from build123d import *

# Parameters (mm, degrees)
SKETCH1_W           = 484
SKETCH1_H           = 378
BOSS_EXTRUDE1_DEPTH = 189
SKETCH2_W           = 318
SKETCH2_H           = 179
CUT_EXTRUDE1_DEPTH  = 553.899629228
SKETCH3_R           = 2.25
SKETCH3_R_2         = 39.056616246
CUT_EXTRUDE2_DEPTH  = 361.563447953


with BuildPart() as part:
    # Sketch1 → Boss-Extrude1 (new body)
    with BuildSketch(Plane(origin=(0, 0, 0), x_dir=(1, 0, 0), z_dir=(0, 1, 0))):
        Rectangle(SKETCH1_W, SKETCH1_H)
    extrude(amount=BOSS_EXTRUDE1_DEPTH)

    # Sketch2 → Cut-Extrude1 (cut, through all)
    with BuildSketch(Plane.ZY.offset(242)):
        with Locations((0, 89.5)):
            Rectangle(SKETCH2_W, SKETCH2_H)
    extrude(amount=-CUT_EXTRUDE1_DEPTH, mode=Mode.SUBTRACT)

    # Sketch3 → Cut-Extrude2 (cut, through all)
    with BuildSketch(Plane(origin=(0, 189, 0), x_dir=(1, 0, 0), z_dir=(0, 1, 0))):
        with Locations(Location((-89, -100, 0), (0, 0, 270))):
            Circle(SKETCH3_R)
        with Locations(Location((89, -100, 0), (0, 0, 270))):
            Circle(SKETCH3_R)
        with Locations(Location((-89, 100, 0), (0, 0, 270))):
            Circle(SKETCH3_R)
        with Locations(Location((89, 100, 0), (0, 0, 270))):
            Circle(SKETCH3_R)
        with Locations(Location((0, 0, 0), (0, 0, 270))):
            Circle(SKETCH3_R_2)
    extrude(amount=-CUT_EXTRUDE2_DEPTH, mode=Mode.SUBTRACT)


solid = part.part
Here's how the part is built. I have some questions about the finished solid (model axes, mm). A direction names the side the tool comes from. Coordinates: 2 decimals unless noted, no trailing zeros. Write each loop counter-clockwise with the first axis right and the second up, starting at its lowest first coordinate (ties: lowest second). Pieces come first, ordered by that corner, then holes.
1) If I drill on line 1 (X direction, y = 182, z = -100); line 2 (Z direction, x = -96, y = 79.5); line 3 (Y direction, x = -42.5, z = -84.5), over which ranges is the centre line in solid material (lowest first)?
Filled in:
line 1: x = -242 to -91.25, -86.75 to 86.75, 91.25 to 242
line 2: z = -189 to -159, 159 to 189
line 3: y = 179 to 189
2) If we section it at D-D (z = -92): List the corners of the cut face in (x, y) for me.
Filled in:
outline: (-242, 179) - (242, 179) - (242, 189) - (-242, 189) - close
3) If we section it at A-A (z = 0): List the corners of the cut face in (x, y) for me, plus the area to 3 significant figures.
Filled in:
outline: (-242, 179) - (-39.06, 179) - (-39.06, 189) - (-242, 189) - close; (39.06, 179) - (242, 179) - (242, 189) - (39.06, 189) - close
area: 4,060 mm2
4) If we section it at B-B (y = 48): List the corners of the cut face in (x, z) for me.
Filled in:
outline: (-242, -189) - (242, -189) - (242, -159) - (-242, -159) - close; (-242, 159) - (242, 159) - (242, 189) - (-242, 189) - close
5) I'm going to push a flat-ended pin straight in: pin 1 (6 mm diameter, centred on x = 19.5, z = -108, fed in from -Y). Where does the tip first touch, or does it pass through?
Filled in:
pin 1: stops at y = 179
6) Thinking about a two-plate mould opening in Z: for faces 3 (the face through (-3, 93, -189)), 4 (the face through (-3, 0, 174)), 5 (the face through (-23.77, 184.07, -30.99)), which applies, +Z half, -Z half, draft (parallel to the pull), parting line (faces both ways), or undercut?
Filled in:
face 3: -Z half
face 4: draft
face 5: undercut
7) Which directions (+Z, -Z, +X, -X, +Y, -Y) give clear straight access to the entire face, cutting with the end or side of a thin tool? Please do faces 1 (the face through (-242, 185, 1)), 2 (the face through (-3, 88, 159)).
Filled in:
face 1: +Z, -Z, -X, +Y, -Y
face 2: +X, -X, -Y
8) If we section it at C-C (x = 128.5): List the corners of the cut face in (y, z) for me, plus the area to 3 significant figures.
Filled in:
outline: (0, -189) - (189, -189) - (189, 189) - (0, 189) - (0, 159) - (179, 159) - (179, -159) - (0, -159) - close
area: 14,500 mm2
